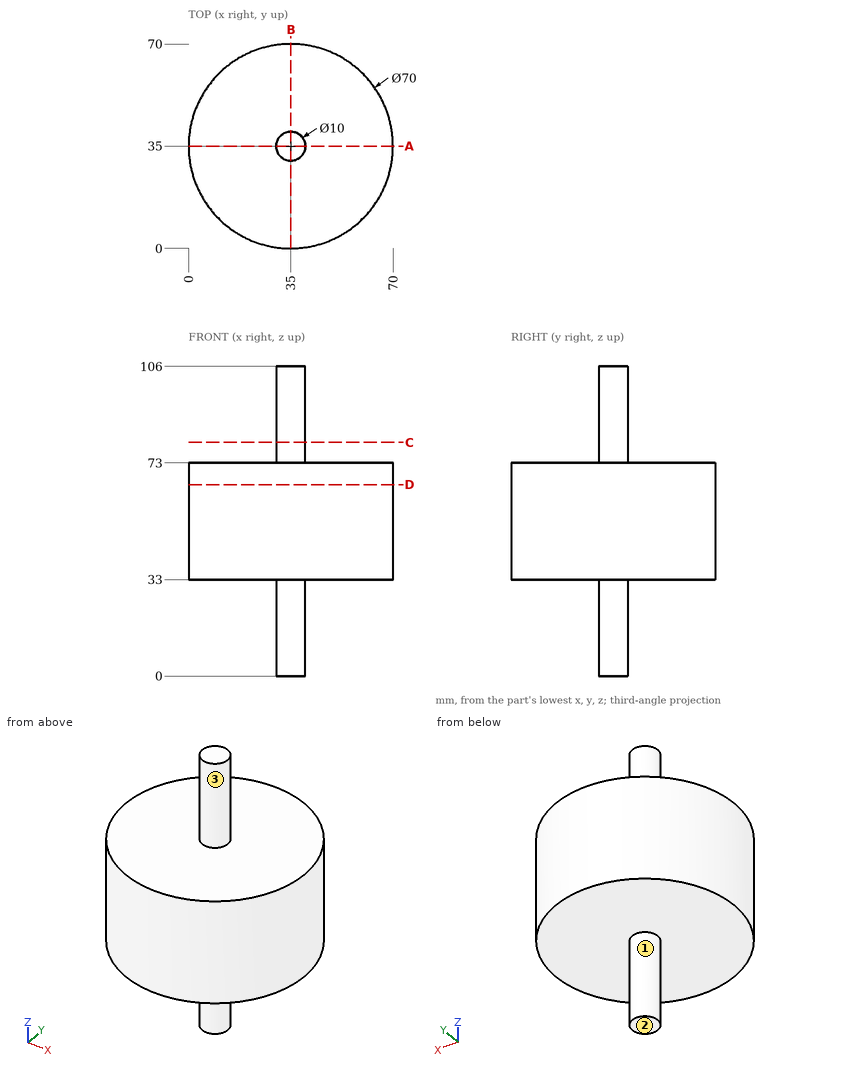
Answer from the drawing. Dimensions are ordinates in mm from the lowest x, y and z of the part. A direction names the side the tool comes from. Give positions to 0.01 mm unless a question says otherwise; leave off trailing zeros. Loops run counter-clockwise (first coordinate to the right, second up) from the corner with the lowest first, then second, coordinate; pieces in that order, holes last. Notation, with made-up numbers: M -28.75,-32.5 L -8.75,-32.5 A26 ccw -8.75,-1.5 Z; hole C 69,15 d5. An arc over 180 degrees is marked long. One line per item, written item: value.
Q1. A cutting plane is placed at D-D on z = 65.5. Determine the outline of the cut face in (x, y), then the cut area to 3 significant figures.
Working result:
outline: C 35,35 d70
area: 3,850 mm^2
Q2. A cutting plane is placed at C-C on z = 80. Determine the outline of the cut face in (x, y), then the cut area to 3 significant figures.
Working result:
outline: C 35,35 d10
area: 78.5 mm^2
Q3. For the marked faces 1, 2 and 3, determine the directions among +Z, -Z, +X, -X, +Y, -Y from which every point of the face is accessible in a straight line to the end or side of a thin tool.
Working result:
face 1: -Z
face 2: -Z, +X, -X, +Y, -Y
face 3: +Z
Q4. Find the intervals of material crossed by line 1 (Z direction, x = 31, y = 62.5); line 2 (Y direction, x = 63, z = 41); line 3 (Y direction, x = 38, z = 54.5), in increasing order. Write a range as from..to.
Working result:
line 1: z = 33..73
line 2: y = 14..56
line 3: y = 0.13..69.87
Q5. A cutting plane is placed at A-A on y = 35. Determine the outline of the cut face in (x, z), then the cut area to 3 significant figures.
Working result:
outline: M 0,33 L 30,33 L 30,0 L 40,0 L 40,33 L 70,33 L 70,73 L 40,73 L 40,106 L 30,106 L 30,73 L 0,73 Z
area: 3,460 mm^2
Q6. Flat-ended cylindrical pins translate along their axes: P1, Ø4, axis at y = 52, z = 55.5, coming from the +X side; P2, Ø5, axis at y = 32, z = 30, coming from the +X side; P3, Ø6, axis at x = 15.5, y = 57.5, coming from the +Z side. Find the tip coordinate at first contact, or state that the pin passes through.
Working result:
P1: stops at x = 66.62
P2: stops at x = 39.97
P3: stops at z = 73
